The listing builds one solid part. Answer for the finished solid, in the listing's coordinates (mm). A direction names the side the tool comes from. Round coordinates to 2 decimals unless told otherwise and drop trailing zeros. Write each loop counter-clockwise with the first axis right and the second up, starting at its lowest first coordinate (ties: lowest second). Pieces come first, ordered by that corner, then holes. Notation, with made-up numbers: (-27, 3) - (0, 3) arc R27 ccw to (0, 21) - close; hole circle Ø11 at (22.5, -36). An arc over 180 degrees is marked (long way). Return JSON: item names as keys, results as strings. Group by question number.
from build123d import *

# Parameters (mm, degrees)
EXTRUDE_1_DEPTH        = 2.5
FILLET_1_R             = 1
FILLET_2_R             = 2.5
FILLET_1_OF_MIRROR_1_R = 1
FILLET_2_OF_MIRROR_1_R = 2.5


with BuildPart() as part:
    # 草图2 → 凸台-拉伸1 (new body)
    with BuildSketch(Plane.XY):
        with BuildLine():
            Line((-4.5, -6.579113924), (-0.5, -6.579113924))
            ThreePointArc((-0.5, -6.579113924), (-0.353553391, -6.225560533), (0, -6.079113924))
            ThreePointArc((0, -6.079113924), (14.918190439, 15.70427557), (-10.784713231, 21.739936821))
            Line((-10.784713231, 21.739936821), (-13.143869251, 24.325354172))
            ThreePointArc((-13.143869251, 24.325354172), (-15.194957506, 22.142312604), (-16.887495374, 19.670886076))
            Line((-16.887495374, 19.670886076), (-10.392304845, 15.920886076))
            ThreePointArc((-10.392304845, 15.920886076), (10.392304845, 15.920886076), (0, -2.079113924))
            ThreePointArc((0, -2.079113924), (-3.181980515, -3.397133409), (-4.5, -6.579113924))
        make_face()
    extrude_1 = extrude(amount=EXTRUDE_1_DEPTH)

    # 圆角1
    fillet_1_edges = [part.edges().sort_by_distance(p)[0] for p in [
        (-10.784713231, 21.739936821, 1.25),
    ]]
    fillet(fillet_1_edges, radius=FILLET_1_R)

    # 圆角2
    fillet_2_edges = [part.edges().sort_by_distance(p)[0] for p in [
        (-10.392304845, 15.920886076, 1.25),
    ]]
    fillet(fillet_2_edges, radius=FILLET_2_R)

    # 镜向1: 凸台-拉伸1 across plane
    add(extrude_1.mirror(Plane.ZX.offset(-6.579113924)))

    # 圆角1 of 镜向1
    fillet_1_of_mirror_1_edges = [part.edges().sort_by_distance(p)[0] for p in [
        (-10.784713231, -34.898164669, 1.25),
    ]]
    fillet(fillet_1_of_mirror_1_edges, radius=FILLET_1_OF_MIRROR_1_R)

    # 圆角2 of 镜向1
    fillet_2_of_mirror_1_edges = [part.edges().sort_by_distance(p)[0] for p in [
        (-10.392304845, -29.079113924, 1.25),
    ]]
    fillet(fillet_2_of_mirror_1_edges, radius=FILLET_2_OF_MIRROR_1_R)


solid = part.part
(1) Determine the mould class of faces 1 (the flat face through (3, -9, 2.5)), 2 (the cylindrical face through (-10.76, -35.29, 1.27)), 3 (the cylindrical face through (15.22, -28.02, 1.23)) for opening direction Y: +Y half, -Y half, draft (parallel to the pull), parting line (faces both ways), or undercut.
(2) Find section C-C (y = 3). Write down the section's boundary in (x, z).
(3) Flat-ended cylindrical pins translate along their axes: pin 1 (1 mm diameter, centred on y = -21, z = 2, fed in from -X); pin 2 (1 mm diameter, centred on y = 0.5, z = 0.5, fed in from +X). Find the tip coordinate at first contact, or state that the pin passes through.
(4) Find section B-B (y = -15.5). Write down the section's boundary in (x, z), plus the area to 3 significant figures.
(5) Find section A-A (z = 1.3). Write down the section's boundary in (x, y).
(6) For faces 4 (the flat face through (-12.279, -36.536, 1.232)), 5 (the flat face through (-14.66, 18.385, 1.232)), 6 (the cylindrical face through (-10.71, 16.76, 1.27)), 7 (the flat face through (-12.3, 23.4, 1.2)), determine the directions among +Z, -Z, +X, -X, +Y, -Y from which every point of the face is accessible in a straight line to the end or side of a thin tool.
(7) Consider line 1 (Y direction, x = 14.5, z = 0.8); line 2 (Y direction, x = -5, z = 2.05); line 3 (Y direction, x = 7.5, z = 1.85). Determine where each line is inside the solid, lowest interval first.
Check sheet entries:
{
 "1": {"face 1": "draft", "face 2": "-Y half", "face 3": "undercut"},
 "2": {"outline": "(9.8, 0) - (14.43, 0) - (14.43, 2.5) - (9.8, 2.5) - close"},
 "3": {"pin 1": "stops at x = 11.72", "pin 2": "stops at x = 13.28"},
 "4": {"outline": "(9.3, 0) - (14.09, 0) - (14.09, 2.5) - (9.3, 2.5) - close", "area": "12.0 mm^2"},
 "5": {"outline": "(-16.89, -32.83) arc R19.5 ccw to (-13.14, -37.48) - (-11.44, -35.62) arc R1 cw to (-10.07, -35.51) arc R16 ccw (long way) to (0, -7.08) arc R0.5 cw to (0, -6.08) arc R16 ccw (long way) to (-10.07, 22.35) arc R1 cw to (-11.44, 22.46) - (-13.14, 24.33) arc R19.5 ccw to (-16.89, 19.67) - (-12.37, 17.06) arc R2.5 ccw to (-9.2, 17.62) arc R12 cw (long way) to (0, -2.08) arc R4.5 ccw to (0, -11.08) arc R12 cw (long way) to (-9.2, -30.78) arc R2.5 ccw to (-12.37, -30.22) - close"},
 "6": {"face 4": "+Z, -Z, -Y", "face 5": "+Z, -Z, -X", "face 6": "+Z, -Z", "face 7": "+Z, -Z, +Y"},
 "7": {"line 1": "y = -29.84 to -16.32, 3.16 to 16.68", "line 2": "y = -38.28 to -33.99, 20.83 to 25.12", "line 3": "y = -37.21 to -32.45, -13.71 to -8.95, -4.21 to 0.55, 19.29 to 24.05"}
}
